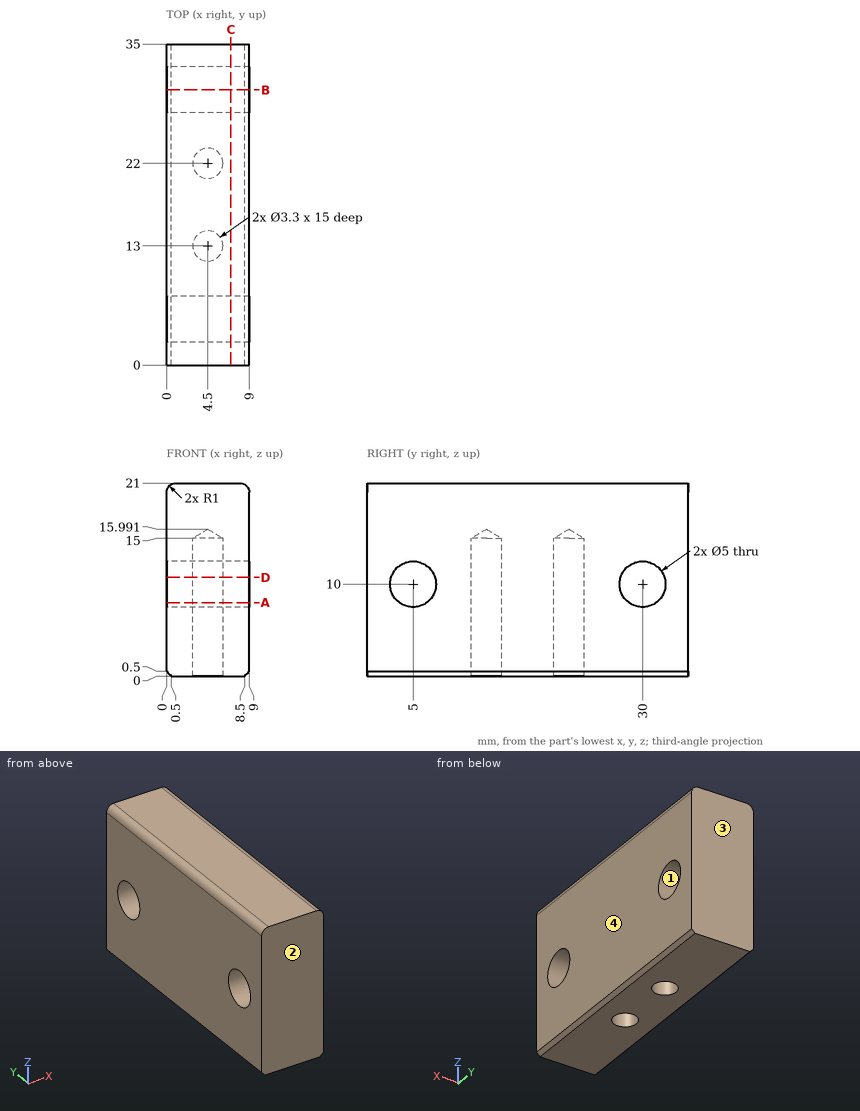
Check sheet for the drawn part. Datum: minimum x, y, z corner. Units: mm. Round coordinates to 2 decimals unless told otherwise and drop trailing zeros. Loops run counter-clockwise (first coordinate to the right, second up) from the corner with the lowest first, then second, coordinate; pieces in that order, holes last. Notation, with made-up numbers: M 11,34.25 L 36,34.25 A20 cw 36,43.25 Z; hole C 57.25,44.25 d1. An arc over 180 degrees is marked long. Write each question's results on one line, items separated by ' | '.
1) Mould release check, pull along Y, two halves, no side actions. Record for the marked faces 1, 2, 3 and 4: released by +Y, released by -Y, zero draft, split by the parting line, or undercut.
Checks:
face 1: undercut | face 2: released by -Y | face 3: released by +Y | face 4: zero draft
2) Section check C-C on x = 7. Record the boundary of the cut face in (y, z).
Checks:
outline: M 0,0 L 35,0 L 35,21 L 0,21 Z; hole C 5,10 d5; hole C 30,10 d5
3) Section check D-D on z = 10.75. State how many separate pieces and enclosed holes the cut face has, then the cut area to 3 significant figures.
Checks:
separate pieces: 3 | enclosed holes: 2 | area: 212 mm2
4) Section check B-B on y = 30. Record the boundary of the cut face in (x, z), then the cut area to 3 significant figures.
Checks:
outline: M 0,0.5 L 0.5,0 L 8.5,0 L 9,0.5 L 9,7.5 L 0,7.5 Z; M 0,12.5 L 9,12.5 L 9,20 A1 ccw 8,21 L 1,21 A1 ccw 0,20 Z | area: 143 mm2
5) Section check A-A on z = 8. Record the boundary of the cut face in (x, y).
Checks:
outline: M 0,0 L 9,0 L 9,3.5 L 0,3.5 Z; M 0,6.5 L 9,6.5 L 9,28.5 L 0,28.5 Z; M 0,31.5 L 9,31.5 L 9,35 L 0,35 Z; hole C 4.5,13 d3.3; hole C 4.5,22 d3.3
6) Scan lines: L1, parallel to Y at x = 2.25, z = 10; L2, parallel to Y at x = 1, z = 9.5; L3, parallel to Y at x = 3.5, z = 8 (1 decimal). Record each from-to range of solid material in increasing order. Write a range as from..to.
Checks:
L1: y = 0..2.5, 7.5..27.5, 32.5..35 | L2: y = 0..2.55, 7.45..27.55, 32.45..35 | L3: y = 0..3.5, 6.5..11.7, 14.3..20.7, 23.3..28.5, 31.5..35
